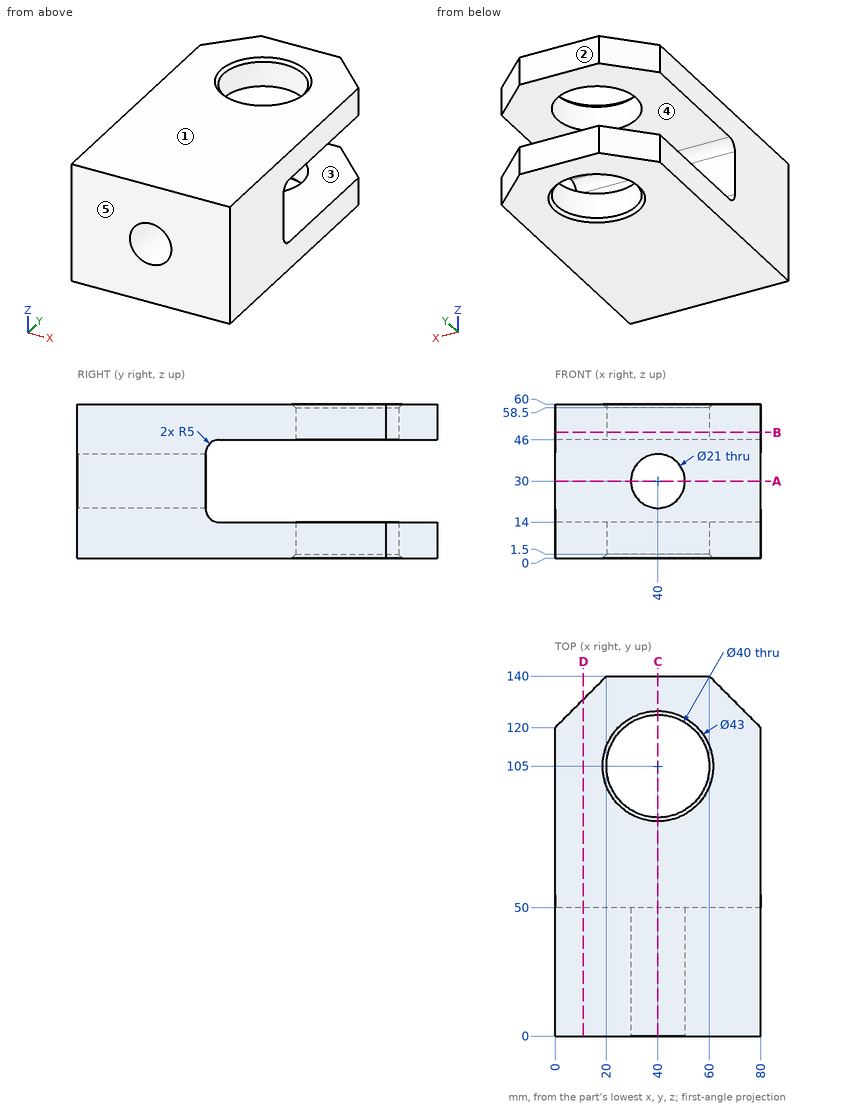
Source: three-view drawing plus pictorial views. Frame: mm from the lowest corner of the part. A direction names the side the tool comes from. Give positions to 0.01 mm unless a question says otherwise; leave off trailing zeros. Order: outer loops, then holes, each group sorted by start corner. A loop starts at its lowest first (then second) coordinate and runs counter-clockwise, first axis right, second up.
1. Material intervals for L1, parallel to Y at x = 40, z = 53; L2, parallel to Z at x = 40, y = 36; L3, parallel to Z at x = 62.5, y = 114, sorted ascending.
Derived:
L1: y = 0 to 85, 125 to 140
L2: z = 0 to 19.5, 40.5 to 60
L3: z = 0 to 14, 46 to 60
2. Section C-C on x = 40. Return the cut outline in (y, z).
Derived:
outline: (0, 0) - (83.5, 0) - (85, 1.5) - (85, 14) - (55, 14) arc R5 cw to (50, 19) - (50, 19.5) - (0, 19.5) - close; (0, 40.5) - (50, 40.5) - (50, 41) arc R5 cw to (55, 46) - (85, 46) - (85, 58.5) - (83.5, 60) - (0, 60) - close; (125, 1.5) - (126.5, 0) - (140, 0) - (140, 14) - (125, 14) - close; (125, 46) - (140, 46) - (140, 60) - (126.5, 60) - (125, 58.5) - close
3. Reachability of the marked faces 4 and 5 from +Z, -Z, +X, -X, +Y, -Y: full face, straight path, thin tool, end or side. Return the list, or none.
Derived:
face 4: +X, -X, +Y
face 5: +Z, -Z, +X, -X, -Y
4. Section B-B on z = 49. Return the cut outline in (x, y).
Derived:
outline: (0, 0) - (80, 0) - (80, 120) - (60, 140) - (20, 140) - (0, 120) - close; hole circle Ø40 at (40, 105)
5. Section A-A on z = 30. Return the cut outline in (x, y), and give its area (3 significant figures).
Derived:
outline: (0, 0) - (29.5, 0) - (29.5, 50) - (0, 50) - close; (50.5, 0) - (80, 0) - (80, 50) - (50.5, 50) - close
area: 2,950 mm2
6. Section D-D on x = 11. Return the cut outline in (y, z), and give its area (3 significant figures).
Derived:
outline: (0, 0) - (131, 0) - (131, 14) - (55, 14) arc R5 cw to (50, 19) - (50, 41) arc R5 cw to (55, 46) - (131, 46) - (131, 60) - (0, 60) - close
area: 5,280 mm2
7. Mould query, pull axis Z, two halves, no side actions, for the marked faces 1, 2 and 3. Classes: released by +Z, released by -Z, zero draft, split by the parting line, or undercut.
Derived:
face 1: released by +Z
face 2: zero draft
face 3: undercut
